from build123d import *

# Parameters (mm, degrees)
SKETCH_1_R          = 2
EXTRUDE_1_DEPTH     = 7
SKETCH_2_R          = 3
EXTRUDE_2_DEPTH     = 4
SKETCH_3_R          = 5
EXTRUDE_3_DEPTH     = 3
CHAMFER_1_SIZE      = 0.5
CHAMFER_2_SIZE      = 0.2
CHAMFER_3_SIZE      = 0.2
CUT_EXTRUDE_1_DEPTH = 3


with BuildPart() as part:
    # 草图1 → 凸台-拉伸1 (new body)
    with BuildSketch(Plane(origin=(0, 0, 0), x_dir=(1, 0, 0), z_dir=(0, 1, 0))):
        with Locations(Location((0, 0, 0), (0, 0, 270))):
            Circle(SKETCH_1_R)
    extrude(amount=EXTRUDE_1_DEPTH)

    # 草图2 → 凸台-拉伸2 (add)
    with BuildSketch(Plane(origin=(0, 7, 0), x_dir=(1, 0, 0), z_dir=(0, 1, 0))):
        with Locations(Location((0, 0, 0), (0, 0, 270))):
            Circle(SKETCH_2_R)
    extrude(amount=EXTRUDE_2_DEPTH)

    # 草图3 → 凸台-拉伸3 (add)
    with BuildSketch(Plane(origin=(0, 11, 0), x_dir=(1, 0, 0), z_dir=(0, 1, 0))):
        with Locations(Location((0, 0, 0), (0, 0, 270))):
            Circle(SKETCH_3_R)
    extrude(amount=EXTRUDE_3_DEPTH)

    # 倒角1
    chamfer_1_edges = [part.edges().sort_by_distance(p)[0] for p in [
        (0, 14, -5),
    ]]
    chamfer(chamfer_1_edges, length=CHAMFER_1_SIZE)

    # 倒角2
    chamfer_2_edges = [part.edges().sort_by_distance(p)[0] for p in [
        (0, 7, -3),
    ]]
    chamfer(chamfer_2_edges, length=CHAMFER_2_SIZE)

    # 倒角3
    chamfer_3_edges = [part.edges().sort_by_distance(p)[0] for p in [
        (0, 0, -2),
    ]]
    chamfer(chamfer_3_edges, length=CHAMFER_3_SIZE)

    # 草图4 → 切除-拉伸1 (cut)
    with BuildSketch(Plane(origin=(0, 14, 0), x_dir=(1, 0, 0), z_dir=(0, 1, 0))):
        Polygon((1.090848991, -1.345380422), (1.710558118, 0.272012727), (0.619709128, 1.617393149), (-1.090848991, 1.345380422), (-1.710558118, -0.272012727), (-0.619709128, -1.617393149), align=None)
    extrude(amount=-CUT_EXTRUDE_1_DEPTH, mode=Mode.SUBTRACT)


solid = part.part
Part model, mm, in its own coordinate system. A direction names the side the tool comes from. Round coordinates to 2 decimals unless told otherwise and drop trailing zeros. Loops run counter-clockwise (first coordinate to the right, second up) from the corner with the lowest first, then second, coordinate; pieces in that order, holes last. Notation, with made-up numbers: (59, 21.5) - (68, 21.5) arc R29 ccw to (68, 57.5) - close; hole circle Ø3 at (44.5, 53). An arc over 180 degrees is marked (long way). Answer as a JSON object with one key per item and string values.
Item 1: Wall check: L1, parallel to Y at x = 2.25, z = -3.5; L2, parallel to X at y = 11.25, z = 1.25; L3, parallel to Z at x = 0.25, y = 12.75. Give the ranges that are in metal, low to high.
Output:
{"L1": "11 to 14", "L2": "-4.84 to -0.92, 1.13 to 4.84", "L3": "-4.99 to -1.56, 1.48 to 4.99"}
Item 2: Tool access for faces 1 (the face through (1.396, 12.521, 0.548)), 2 (the face through (-3.3, 11, -0.1)), 3 (the face through (-2, 14, 0)): list every direction of +Z, -Z, +X, -X, +Y, -Y with a clear straight run to the whole face (end or side of a thin tool).
Output:
{"face 1": "+Y", "face 2": "-Y", "face 3": "+Z, -Z, +X, -X, +Y"}
Item 3: Band-saw the part on A-A on y = 9.5. List the corners of the cut face in (x, z).
Output:
{"outline": "circle Ø6 at (0, 0)"}
Item 4: Pin check, flat tips, straight feed: pin 1 (1 mm diameter, centred on x = -0.5, z = 0.5, fed in from +Y); pin 2 (2 mm diameter, centred on y = 9.5, z = -0.5, fed in from +X); pin 3 (5 mm diameter, centred on x = 0, y = 2.5, fed in from -Z). Stop position of each tip, or through.
Output:
{"pin 1": "y = 11", "pin 2": "x = 3", "pin 3": "z = -2"}
Item 5: Band-saw the part on B-B on x = 0. List the corners of the cut face in (y, z).
Output:
{"outline": "(0, -1.8) - (0.2, -2) - (7, -2) - (7, -2.8) - (7.2, -3) - (11, -3) - (11, -5) - (13.5, -5) - (14, -4.5) - (14, -1.52) - (11, -1.52) - (11, 1.52) - (14, 1.52) - (14, 4.5) - (13.5, 5) - (11, 5) - (11, 3) - (7.2, 3) - (7, 2.8) - (7, 2) - (0.2, 2) - (0, 1.8) - close"}
Item 6: Band-saw the part on D-D on y = 3.75. List the corners of the cut face in (x, z), plus the area to 3 significant figures.
Output:
{"outline": "circle Ø4 at (0, 0)", "area": "12.6 mm2"}
Item 7: Pull direction X, two halves, no side cores. Call faces 4 (the face through (0, 0, 0)), 5 (the face through (-4.88, 12.23, -1.08)), 6 (the face through (-1.2, 12.5, 0.9)): pulls with the +X half, pulls with the -X half, needs draft (parallel to the pull), parting line crosses it, or undercut.
Output:
{"face 4": "needs draft", "face 5": "parting line crosses it", "face 6": "undercut"}
Item 8: Band-saw the part on C-C on z = 0. List the corners of the cut face in (x, y).
Output:
{"outline": "(-5, 11) - (-3, 11) - (-3, 7.2) - (-2.8, 7) - (-2, 7) - (-2, 0.2) - (-1.8, 0) - (1.8, 0) - (2, 0.2) - (2, 7) - (2.8, 7) - (3, 7.2) - (3, 11) - (5, 11) - (5, 13.5) - (4.5, 14) - (1.61, 14) - (1.61, 11) - (-1.61, 11) - (-1.61, 14) - (-4.5, 14) - (-5, 13.5) - close"}
